from build123d import *

# Parameters (mm, degrees)
BOSS_EXTRUDE1_DEPTH = 6.4
SKETCH4_R           = 17.59
SKETCH4_R_2         = 8
CUT_EXTRUDE1_DEPTH  = 0.8
CUT_EXTRUDE1_DRAFT  = -60
CHAMFER2_SIZE       = 0.555555556


with BuildPart() as part:
    # Sketch3 → Boss-Extrude1 (new body)
    with BuildSketch(Plane(origin=(0, 0, 0), x_dir=(0, 0, -1), z_dir=(1, 0, 0))):
        Polygon((8, 4.618802154), (0, 9.237604307), (-8, 4.618802154), (-8, -4.618802154), (0, -9.237604307), (8, -4.618802154), align=None)
    extrude(amount=BOSS_EXTRUDE1_DEPTH)


with BuildPart() as cut_extrude1_tool:
    # Sketch4 → Cut-Extrude1 (with draft: the straight prism first)
    with BuildSketch(Plane.ZY):
        Circle(SKETCH4_R)
        Circle(SKETCH4_R_2, mode=Mode.SUBTRACT)
    extrude(amount=-CUT_EXTRUDE1_DEPTH)
    # Cut-Extrude1: the draft: its side faces are tilted about the plane it starts from
    cut_extrude1_sides = [cut_extrude1_tool.faces().sort_by_distance(p)[0] for p in [
        (0.4, 0, -17.59),
        (0.4, 0, -8),
    ]]
    draft(cut_extrude1_sides, Plane.ZY, CUT_EXTRUDE1_DRAFT)


with BuildPart() as part_1:
    add(part.part)

    # Cut-Extrude1: cut by cut_extrude1_tool
    add(cut_extrude1_tool.part, mode=Mode.SUBTRACT)

    # Sketch5 → Revolve1 (revolve)
    with BuildSketch(Plane.XY, mode=Mode.PRIVATE) as revolve1_sk:
        with BuildLine():
            Line((7.5, 5), (46.4, 5))
            Line((46.4, 5), (46.4, 0))
            Line((46.4, 0), (6.4, 0))
            Line((6.4, 0), (6.4, 6.1))
            ThreePointArc((6.4, 6.1), (6.722182541, 5.322182541), (7.5, 5))
        make_face()
    revolve(revolve1_sk.sketch.rotate(Axis((6.4, 0, 0), (1, 0, 0)), 90), axis=Axis((6.4, 0, 0), (1, 0, 0)))

    # Chamfer2
    chamfer2_edges = [part_1.edges().sort_by_distance(p)[0] for p in [
        (46.4, 0, -5),
    ]]
    chamfer(chamfer2_edges, length=CHAMFER2_SIZE)


solid = part_1.part
Can you work these out from the model? Positions are in its coordinate system, mm. A direction names the side the tool comes from. Round coordinates to 2 decimals unless told otherwise and drop trailing zeros. Order: outer loops, then holes, each group sorted by start corner. A loop starts at its lowest first (then second) coordinate and runs counter-clockwise, first axis right, second up. Notation, with made-up numbers: (21.5, 22) - (58.5, 22) arc R11 ccw to (58.5, 37) - close; hole circle Ø8 at (7.5, 75.5). An arc over 180 degrees is marked (long way). Answer in a Markdown table with one row per item.
(1) Which directions (+Z, -Z, +X, -X, +Y, -Y) give clear straight access to the entire face, cutting with the end or side of a thin tool? Please do faces 1 (the face through (0, 0, 0)), 2 (the face through (6.4, -4, -5)).
From the geometry:
| item | result |
|---|---|
| face 1 | +Z, -Z, -X, +Y, -Y |
| face 2 | +X |
(2) For P1, Ø8, axis at x = 39, z = 4, coming from the +Y side; P2, Ø3, axis at x = 39.5, y = -0.5, coming from the +Z side; P3, Ø6, axis at x = 13.5, y = 5.5, coming from the +Z side, each with a flat end and sliding along its axis, tell me the tip position at first contact or that it passes through.
From the geometry:
| item | result |
|---|---|
| P1 | stops at y = 5 |
| P2 | stops at z = 5 |
| P3 | stops at z = 4.33 |
(3) Please list where these lines run through material, in increasing order: L1, parallel to X at y = 4.25, z = -5.5; L2, parallel to Y at x = 40, z = -3. Write a range as from..to.
From the geometry:
| item | result |
|---|---|
| L1 | x = 0..6.4 |
| L2 | y = -4..4 |
(4) Suppose I cut it at A-A, the plane x = 35.5. Please give me the cut outline in (y, z), plus the area to 3 significant figures.
From the geometry:
| item | result |
|---|---|
| outline | circle Ø10 at (0, 0) |
| area | 78.5 mm2 |
